from build123d import *

# Parameters (mm, degrees)
SKETCH_1_R          = 22.5
EXTRUDE_1_DEPTH     = 2
SKETCH_2_R          = 20
SKETCH_2_R_2        = 17.5
EXTRUDE_2_DEPTH     = 11
SKETCH_3_R          = 7.678665591
CUT_EXTRUDE_1_DEPTH = 21


with BuildPart() as part:
    # 草图1 → 凸台-拉伸1 (new, symmetric)
    with BuildSketch(Plane.XY):
        Circle(SKETCH_1_R)
    extrude(amount=EXTRUDE_1_DEPTH, both=True)

    # 草图2 → 凸台-拉伸2 (add)
    with BuildSketch(Plane.XY.offset(2)):
        Circle(SKETCH_2_R)
        Circle(SKETCH_2_R_2, mode=Mode.SUBTRACT)
    extrude(amount=EXTRUDE_2_DEPTH)

    # 草图3 → 切除-拉伸1 (cut)
    with BuildSketch(Plane.XY.offset(2)):
        Circle(SKETCH_3_R)
    extrude(amount=-CUT_EXTRUDE_1_DEPTH, mode=Mode.SUBTRACT)


solid = part.part
Geometry check sheet. Reference: the model listing, model coordinates, mm. A direction names the side the tool comes from. Give positions to 0.01 mm unless a question says otherwise; leave off trailing zeros. Write each loop counter-clockwise with the first axis right and the second up, starting at its lowest first coordinate (ties: lowest second). Pieces come first, ordered by that corner, then holes. Notation, with made-up numbers: (-33, 19) - (18, 19) arc R23 ccw to (18, 56) - close; hole circle Ø6 at (27.25, -31.5). An arc over 180 degrees is marked (long way). Put each result on its own line as item: value.
1. Draft check along Y on faces 1 (the cylindrical face through (-13.887, -10.648, 7.423)), 2 (the flat face through (-20.1, -1.6, 2)), 3 (the cylindrical face through (-4.336, -19.524, 7.423)). Enter one of: +Y half, -Y half, draft (parallel to the pull), parting line (faces both ways), or undercut.
Ans:
face 1: undercut
face 2: draft
face 3: parting line
2. Sectioned sample at A-A, the plane x = 0. Enter the section's corners in (y, z).
Ans:
outline: (-22.5, -2) - (-7.68, -2) - (-7.68, 2) - (-17.5, 2) - (-17.5, 13) - (-20, 13) - (-20, 2) - (-22.5, 2) - close; (7.68, -2) - (22.5, -2) - (22.5, 2) - (20, 2) - (20, 13) - (17.5, 13) - (17.5, 2) - (7.68, 2) - close
3. Sectioned sample at C-C, the plane z = 10. Enter the section's corners in (x, y), plus the area to 3 significant figures.
Ans:
outline: circle Ø40 at (0, 0); hole circle Ø35 at (0, 0)
area: 295 mm²
4. Thickness scan on line 1 (Y direction, x = 0, z = -0.8); line 2 (Y direction, x = 0, z = 4.5); line 3 (Z direction, x = 2, y = -14). Record the ranges inside material, lowest first.
Ans:
line 1: y = -22.5 to -7.68, 7.68 to 22.5
line 2: y = -20 to -17.5, 17.5 to 20
line 3: z = -2 to 2
5. Set-up check for faces 4 (the flat face through (0, -18, 13)), 5 (the flat face through (4, -8, 2)): record each of +Z, -Z, +X, -X, +Y, -Y from which the full face is reachable in a straight line by a thin tool's end or side.
Ans:
face 4: +Z, +X, -X, +Y, -Y
face 5: +Z
6. Sectioned sample at D-D, the plane x = 10. Enter the section's corners in (y, z), plus the area to 3 significant figures.
Ans:
outline: (-20.16, -2) - (20.16, -2) - (20.16, 2) - (17.32, 2) - (17.32, 13) - (14.36, 13) - (14.36, 2) - (-14.36, 2) - (-14.36, 13) - (-17.32, 13) - (-17.32, 2) - (-20.16, 2) - close
area: 226 mm²
7. Go/stop test with flat-tipped pins: pin 1 (6 mm diameter, centred on y = 10.5, z = 1, fed in from -X); pin 2 (3 mm diameter, centred on x = 12.5, z = 1, fed in from -Y); pin 3 (4 mm diameter, centred on y = 4.5, z = 4.5, fed in from +X). Record where each tip stops, or that it passes through.
Ans:
pin 1: stops at x = -21.21
pin 2: stops at y = -19.63
pin 3: stops at x = 19.84
